from build123d import *

# Parameters (mm, degrees)
CUT_EXTRUDE1_DEPTH  = 15
SKETCH4_R           = 10.25
CUT_EXTRUDE2_DEPTH  = 3.5
SKETCH5_R           = 1.75
CUT_EXTRUDE3_DEPTH  = 5
SKETCH7_R           = 20
SKETCH7_R_2         = 1.75
SKETCH7_R_3         = 9
BOSS_EXTRUDE1_DEPTH = 3
CUT_EXTRUDE5_REACH  = 36.321
SKETCH10_R          = 1.65
CHAMFER1_SIZE       = 0.3
CHAMFER2_SIZE       = 0.3


with BuildPart() as part:
    # Sketch1 → Revolve1 (revolve)
    with BuildSketch(Plane.XY, mode=Mode.PRIVATE) as revolve1_sk:
        Polygon((0, 9), (0, 14), (15, 14), (15, 22), (20, 22), (20, 9), align=None)
    revolve(revolve1_sk.sketch.rotate(Axis((0, 0, 0), (1, 0, 0)), 90), axis=Axis((0, 0, 0), (1, 0, 0)))

    # Sketch3 → Cut-Extrude1 (cut, symmetric)
    with BuildSketch(Plane.XY):
        Polygon((9.613311632, 17.562947239), (8.386688368, -17.562947239), (-5.415654366, -17.562947239), (-5.415654366, 17.562947239), align=None)
    extrude(amount=CUT_EXTRUDE1_DEPTH, both=True, mode=Mode.SUBTRACT)

    # Sketch4 → Cut-Extrude2 (cut)
    with BuildSketch(Plane(origin=(8.989038226, -0.313904132, 0), x_dir=(0, 0, 1), z_dir=(-0.9993908270190958, 0.03489949670250087, 0))):
        with Locations(Location((0, 0, 0), (0, 0, 270))):
            Circle(SKETCH4_R)
    extrude(amount=-CUT_EXTRUDE2_DEPTH, mode=Mode.SUBTRACT)

    # Sketch5 → Cut-Extrude3 (cut)
    with BuildSketch(Plane.ZY.offset(-15)):
        with Locations((-17.5, 0)):
            Circle(SKETCH5_R)
        with Locations((0, 17.5)):
            Circle(SKETCH5_R)
        with Locations((17.5, 0)):
            Circle(SKETCH5_R)
        with Locations((0, -17.5)):
            Circle(SKETCH5_R)
    extrude(amount=-CUT_EXTRUDE3_DEPTH, mode=Mode.SUBTRACT)

    # Sketch7 → Boss-Extrude1 (add)
    with BuildSketch(Plane(origin=(20, 0, 0), x_dir=(0, 0, -1), z_dir=(1, 0, 0))):
        with Locations(Location((0, 0, 0), (0, 0, 180))):
            Circle(SKETCH7_R)
        with Locations(Location((17.5, 0, 0), (0, 0, 180))):
            Circle(SKETCH7_R_2, mode=Mode.SUBTRACT)
        with Locations(Location((0, -17.5, 0), (0, 0, 180))):
            Circle(SKETCH7_R_2, mode=Mode.SUBTRACT)
        with Locations(Location((-17.5, 0, 0), (0, 0, 180))):
            Circle(SKETCH7_R_2, mode=Mode.SUBTRACT)
        with Locations(Location((0, 17.5, 0), (0, 0, 180))):
            Circle(SKETCH7_R_2, mode=Mode.SUBTRACT)
        with Locations(Location((0, 0, 0), (0, 0, 270))):
            Circle(SKETCH7_R_3, mode=Mode.SUBTRACT)
    extrude(amount=BOSS_EXTRUDE1_DEPTH)

    # Sketch10 → Cut-Extrude5 (cut, up to next)
    with BuildSketch(Plane(origin=(23, 0, 0), x_dir=(0, 0, -1), z_dir=(1, 0, 0)), mode=Mode.PRIVATE) as cut_extrude5_sk1:
        with Locations((-12.5, 11)):
            Circle(SKETCH10_R)
    cut_extrude5_tool1 = extrude(cut_extrude5_sk1.sketch, amount=-CUT_EXTRUDE5_REACH, mode=Mode.PRIVATE) & part.part
    add(cut_extrude5_tool1.solids().sort_by_distance((23, 11, 12.5))[0], mode=Mode.SUBTRACT)

    # Chamfer1
    chamfer1_edges = [part.edges().sort_by_distance(p)[0] for p in [
        (23, 0, -20),
        (15, 0, -22),
    ]]
    chamfer(chamfer1_edges, length=CHAMFER1_SIZE)

    # Chamfer2
    chamfer2_edges = [part.edges().sort_by_distance(p)[0] for p in [
        (23, 9, 0),
    ]]
    chamfer(chamfer2_edges, length=CHAMFER2_SIZE)


solid = part.part
Input: part model. Units: mm. Frame: model coordinates. A direction names the side the tool comes from. Coordinates: 2 decimals unless noted, no trailing zeros. Loops run counter-clockwise (first coordinate to the right, second up) from the corner with the lowest first, then second, coordinate; pieces in that order, holes last.
(1) Set-up query: faces 1 (the face through (11.75, -13.88, -1.82)), 2 (the face through (17.683, 21.477, -4.769)), 3 (the face through (20, 18, 10)). Return all of +Z, -Z, +X, -X, +Y, -Y with unobstructed straight access to the full face (end or side cutting, diameter ignored); none if empty.
(2) Section B-B on z = 0. Count the separate pieces of the cut face and the enclosed holes in it, then the cut area to 3 significant figures.
(3) First-contact query: pin 1 Ø2 at (y, z) = (0, -17.5) entering from +X; pin 2 Ø23.5 at (y, z) = (0, 0) entering from -X; pin 3 Ø8 at (x, z) = (17.5, -6.5) entering from +Y; pin 4 Ø10 at (y, z) = (14.5, 16) entering from -X. Flat tips, straight axial feed; report the tip coordinate or a pass-through.
(4) Pull-direction query (Z, two-part tool) for faces 4 (the face through (10.997, 7.755, -6.237)), 5 (the face through (23, -4.7, 8.5)), 6 (the face through (21.33, -0.88, -19.98)); classes: released by +Z, released by -Z, zero draft, split by the parting line, or undercut.
(5) Section A-A on x = 21. Return the cut outline in (y, z), then the cut area to 3 significant figures.
(6) Material intervals for probe 1 along Y at (x, z) = (16.6, 0); probe 2 along Z at (x, y) = (16, 1); probe 3 along X at (y, z) = (17.5, -11.5), sorted ascending.
Data:
1. face 1: -X
1. face 2: +X, -X
1. face 3: +X
2. separate pieces: 4
2. enclosed holes: 0
2. area: 191 mm2
3. pin 1: passes through
3. pin 2: stops at x = 8.59
3. pin 3: stops at y = 21.86
3. pin 4: stops at x = 15
4. face 4: undercut
4. face 5: zero draft
4. face 6: split by the parting line
5. outline: circle Ø40 at (0, 0); hole circle Ø3.5 at (-17.5, 0); hole circle Ø18 at (0, 0); hole circle Ø3.5 at (0, -17.5); hole circle Ø3.5 at (0, 17.5); hole circle Ø3.3 at (11, 12.5); hole circle Ø3.5 at (17.5, 0)
5. area: 955 mm2
6. probe 1: y = -22 to -19.25, -15.75 to -9, 9 to 15.75, 19.25 to 22
6. probe 2: z = -21.98 to -18.94, -16.06 to -8.94, 8.94 to 16.06, 18.94 to 21.98
6. probe 3: x = 15 to 20
